Verification items for the finished model (mm, model axes). Face numbers are marked on the shaded views. A direction names the side the tool comes from. Coordinates: 2 decimals unless noted, no trailing zeros. Order: outer loops, then holes, each group sorted by start corner. A loop starts at its lowest first (then second) coordinate and runs counter-clockwise, first axis right, second up. Notation, with made-up numbers: M 46.5,61.25 L 89.5,61.25 A11 cw 89.5,70.25 Z; hole C -26.75,45.25 d4. An arc over 180 degrees is marked long. Return JSON: item names as keys, results as strings. Group by question number.
1. Gauge pin test, flat ends, axial feed: pin 1 (2 mm diameter, centred on x = -3.35, y = -0.36, fed in from -Z); pin 2 (4 mm diameter, centred on x = 11.65, y = -0.36, fed in from -Z); pin 3 (2 mm diameter, centred on x = -2.5, y = 0, fed in from +Z). Record the tip position at first contact, or that the pin passes through.
2. Mould release check, pull along X, two halves, no side actions. Record for the marked faces 3, 4 and 5: +X half, -X half, draft (parallel to the pull), parting line (faces both ways), or undercut.
3. Section check B-B, the plane z = 4.35. Record the cut outline in (x, y), plus the area to 3 significant figures.
4. Material ranges on line 1 along X through (y, z) = (-0.25, 0.45); line 2 along X through (y, z) = (-1.25, 3.8); line 3 along Y through (x, z) = (-2.5, 4.55), recorded low to high.
5. Section check A-A, the plane y = -1. Record the cut outline in (x, z).
6. Set-up check for the marked faces 1 and 2: record each of +Z, -Z, +X, -X, +Y, -Y from which the full face is reachable in a straight line by a thin tool's end or side.
7. Section check C-C, the plane x = -4. Record the cut outline in (y, z).
8. Section check D-D, the plane y = 1.5. Record the cut outline in (x, z), plus the area to 3 significant figures.
```python
from build123d import *

# Parameters (mm, degrees)
SKETCH_1_W          = 25
SKETCH_1_H          = 6.8
EXTRUDE_1_DEPTH     = 5
CUT_EXTRUDE_1_REACH = 19.791
SKETCH_2_R          = 1.2
SKETCH_3_R          = 2.15
CUT_EXTRUDE_2_DEPTH = 2.4


with BuildPart() as part:
    # 草图1 → 凸台-拉伸1 (new body)
    with BuildSketch(Plane.XY):
        with Locations((4.154545455, -0.360606061)):
            Rectangle(SKETCH_1_W, SKETCH_1_H)
    extrude(amount=EXTRUDE_1_DEPTH)

    # 草图2 → 切除-拉伸1 (cut, up to next)
    with BuildSketch(Plane.XY.offset(5), mode=Mode.PRIVATE) as cut_extrude_1_sk1:
        with Locations((-3.345454545, -0.360606061)):
            Circle(SKETCH_2_R)
    cut_extrude_1_tool1 = extrude(cut_extrude_1_sk1.sketch, amount=-CUT_EXTRUDE_1_REACH, mode=Mode.PRIVATE) & part.part
    # 草图2 → 切除-拉伸1 (cut, up to next)
    with BuildSketch(Plane.XY.offset(5), mode=Mode.PRIVATE) as cut_extrude_1_sk2:
        with Locations((11.654545455, -0.360606061)):
            Circle(SKETCH_2_R)
    cut_extrude_1_tool2 = extrude(cut_extrude_1_sk2.sketch, amount=-CUT_EXTRUDE_1_REACH, mode=Mode.PRIVATE) & part.part
    add(cut_extrude_1_tool1.solids().sort_by_distance((-3.345455, -0.360606, 5))[0], mode=Mode.SUBTRACT)
    add(cut_extrude_1_tool2.solids().sort_by_distance((11.654545, -0.360606, 5))[0], mode=Mode.SUBTRACT)

    # 草图3 → 切除-拉伸2 (cut)
    with BuildSketch(Plane.XY.offset(5)):
        with Locations((-3.345454545, -0.360606061)):
            Circle(SKETCH_3_R)
        with Locations((11.654545455, -0.360606061)):
            Circle(SKETCH_3_R)
    extrude(amount=-CUT_EXTRUDE_2_DEPTH, mode=Mode.SUBTRACT)


solid = part.part
```
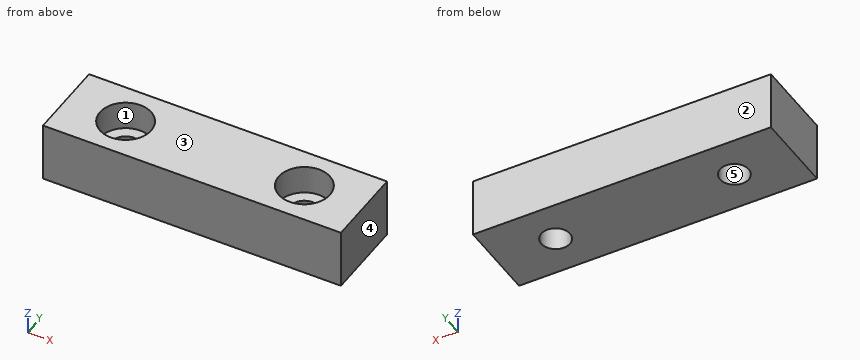
Answers follow:
{
 "1": {"pin 1": "through", "pin 2": "z = 0", "pin 3": "z = 2.6"},
 "2": {"face 3": "draft", "face 4": "+X half", "face 5": "undercut"},
 "3": {"outline": "M -8.35,-3.76 L 16.65,-3.76 L 16.65,3.04 L -8.35,3.04 Z; hole C -3.35,-0.36 d4.3; hole C 11.65,-0.36 d4.3", "area": "141 mm^2"},
 "4": {"line 1": "-8.35 to -4.54, -2.15 to 10.46, 12.85 to 16.65", "line 2": "-8.35 to -5.3, -1.39 to 9.7, 13.61 to 16.65", "line 3": "-3.76 to -2.34, 1.62 to 3.04"},
 "5": {"outline": "M -8.35,0 L -4.36,0 L -4.36,2.6 L -5.4,2.6 L -5.4,5 L -8.35,5 Z; M -2.33,0 L 10.64,0 L 10.64,2.6 L 9.6,2.6 L 9.6,5 L -1.29,5 L -1.29,2.6 L -2.33,2.6 Z; M 12.67,0 L 16.65,0 L 16.65,5 L 13.71,5 L 13.71,2.6 L 12.67,2.6 Z"},
 "6": {"face 1": "+Z", "face 2": "+Z, -Z, +X, -X, +Y"},
 "7": {"outline": "M -3.76,0 L -1.37,0 L -1.37,2.6 L -2.41,2.6 L -2.41,5 L -3.76,5 Z; M 0.65,0 L 3.04,0 L 3.04,5 L 1.69,5 L 1.69,2.6 L 0.65,2.6 Z"},
 "8": {"outline": "M -8.35,0 L 16.65,0 L 16.65,5 L 12.73,5 L 12.73,2.6 L 10.58,2.6 L 10.58,5 L -2.27,5 L -2.27,2.6 L -4.42,2.6 L -4.42,5 L -8.35,5 Z", "area": "115 mm^2"}
}
